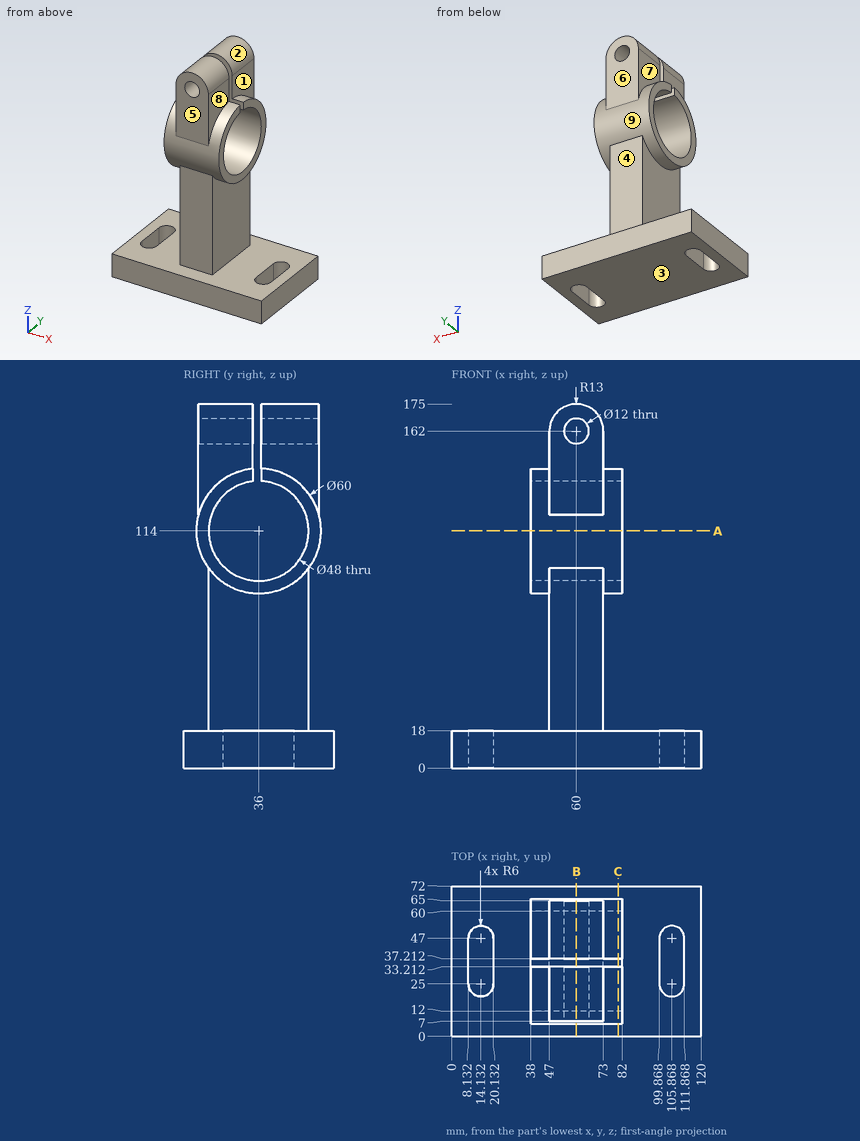
Check sheet for the drawn part. Datum: minimum x, y, z corner. Units: mm. A direction names the side the tool comes from. Coordinates: 2 decimals unless noted, no trailing zeros. Loops run counter-clockwise (first coordinate to the right, second up) from the corner with the lowest first, then second, coordinate; pieces in that order, holes last. Notation, with made-up numbers: (23.5, 4.25) -> (68.5, 4.25) arc R13 cw to (68.5, 28.25) -> close; hole circle Ø2 at (31.5, -14.5). An arc over 180 degrees is marked (long way). Answer in a Markdown table with one row per item.
1) Section check B-B (x = 60). Record the cut outline in (y, z), and give its area (3 significant figures).
The answers:
| item | result |
|---|---|
| outline | (0, 0) -> (72, 0) -> (72, 18) -> (60, 18) -> (60, 96) arc R30 ccw to (65, 121.68) -> (65, 156) -> (37.21, 156) -> (37.21, 137.97) arc R24 cw (long way) to (33.21, 137.84) -> (33.21, 156) -> (7, 156) -> (7, 121.68) arc R30 ccw to (12, 96) -> (12, 18) -> (0, 18) -> close; (7, 168) -> (33.21, 168) -> (33.21, 175) -> (7, 175) -> close; (37.21, 168) -> (65, 168) -> (65, 175) -> (37.21, 175) -> close |
| area | 6,990 mm2 |
2) Access from +Z, -Z, +X, -X, +Y, -Y to the whole of each face (thin tool, end or side, straight path). Record for the marked faces 5, 6, 7, 8 and 9.
The answers:
| item | result |
|---|---|
| face 5 | +Z, +X, -X, -Y |
| face 6 | +Z, +X, -X, +Y |
| face 7 | +Z, -X, +Y |
| face 8 | +Z, +X, -Y |
| face 9 | none |
3) Section check A-A (z = 114). Record the cut outline in (x, y).
The answers:
| item | result |
|---|---|
| outline | (38, 6) -> (82, 6) -> (82, 12) -> (38, 12) -> close; (38, 60) -> (82, 60) -> (82, 66) -> (38, 66) -> close |
4) Scan lines: line 1 along X through (y, z) = (19, 162); line 2 along Z through (x, y) = (42.5, 43); line 3 along Z through (x, y) = (56, 43) (1 decimal). Record each from-to range of solid material in increasing order. Write a range as from..to.
The answers:
| item | result |
|---|---|
| line 1 | x = 47..54, 66..73 |
| line 2 | z = 0..18, 84.83..91.04, 136.96..143.17 |
| line 3 | z = 0..91, 137..157.5, 166.5..174.4 |
5) Depth check by flat-ended pin: P1, Ø21.5, axis at x = 31.5, y = 26.5, coming from the +Z side; P2, Ø21, axis at x = 64.5, z = 76.5, coming from the +Y side; P3, Ø1, axis at y = 58.5, z = 84.5, coming from the -X side. Enter the tip coordinate at first touch or a pass-through.
The answers:
| item | result |
|---|---|
| P1 | stops at z = 143.87 |
| P2 | stops at y = 60 |
| P3 | stops at x = 47 |
6) Section check C-C (x = 80). Record the cut outline in (y, z) (1 decimal), and give its area (3 significant figures).
The answers:
| item | result |
|---|---|
| outline | (0, 0) -> (72, 0) -> (72, 18) -> (0, 18) -> close; (33.2, 137.8) -> (33.2, 143.9) arc R30 ccw (long way) to (37.2, 144) -> (37.2, 138) arc R24 cw (long way) to start |
| area | 2,290 mm2 |
7) Draft check along Z on the marked faces 1, 2, 3 and 4. Enter one of: released by +Z, released by -Z, zero draft, split by the parting line, or undercut.
The answers:
| item | result |
|---|---|
| face 1 | zero draft |
| face 2 | released by +Z |
| face 3 | released by -Z |
| face 4 | undercut |
